from build123d import *

# Parameters (mm, degrees)
SKETCH1_W               = 10.85
SKETCH1_H               = 10.85
BOSS_EXTRUDE1_DEPTH     = 700
MIRROR2_COPY_1_SKETCH_W = 10.85
MIRROR2_COPY_1_SKETCH_H = 10.85
MIRROR2_COPY_1_DEPTH    = 700


with BuildPart() as part:
    # Sketch1 → Boss-Extrude1 (new body)
    with BuildSketch(Plane(origin=(0, 0, 0), x_dir=(1, 0, 0), z_dir=(0, 1, 0))):
        with BuildLine():
            Line((-4.3, 20), (-19.5, 20))
            ThreePointArc((-19.5, 20), (-19.853553391, 19.853553391), (-20, 19.5))
            Line((-20, 19.5), (-20, 4.3))
            Line((-20, 4.3), (-19.05, 4.3))
            Line((-19.05, 4.3), (-19.05, 7.25))
            Line((-19.05, 7.25), (-7.921751442, 7.25))
            Line((-7.921751442, 7.25), (-6.2, 5.528248558))
            Line((-6.2, 5.528248558), (-6.2, 0))
            Line((-6.2, 0), (-5.3, 0))
            ThreePointArc((-5.3, 0), (-5.066731596, 1.555066215), (-4.387460025, 2.973246463))
            Line((-4.387460025, 2.973246463), (-5.091168825, 3.676955262))
            ThreePointArc((-5.091168825, 3.676955262), (-5.091168825, 5.091168825), (-3.676955262, 5.091168825))
            Line((-3.676955262, 5.091168825), (-2.973246463, 4.387460025))
            ThreePointArc((-2.973246463, 4.387460025), (-1.555066215, 5.066731596), (0, 5.3))
            Line((0, 5.3), (0, 6.2))
            Line((0, 6.2), (-5.528248558, 6.2))
            Line((-5.528248558, 6.2), (-7.25, 7.921751442))
            Line((-7.25, 7.921751442), (-7.25, 19.05))
            Line((-7.25, 19.05), (-4.3, 19.05))
            Line((-4.3, 19.05), (-4.3, 20))
        make_face()
        with Locations((-13.625, 13.625)):
            Rectangle(SKETCH1_W, SKETCH1_H, mode=Mode.SUBTRACT)
    boss_extrude1 = extrude(amount=BOSS_EXTRUDE1_DEPTH)

    # Mirror1: Boss-Extrude1 across plane
    add(boss_extrude1.mirror(Plane(origin=(0, 0, 0), x_dir=(0, 0, 1), z_dir=(1, 0, 0))))

    # Mirror2: Boss-Extrude1 across plane
    add(boss_extrude1.mirror(Plane.XY))

    # Mirror2 copy 1 sketch → Mirror2 copy 1 (add)
    with BuildSketch(Plane(origin=(0, 0, 0), x_dir=(-1, 0, 0), z_dir=(0, 1, 0))):
        with BuildLine():
            Line((-4.3, 20), (-19.5, 20))
            ThreePointArc((-19.5, 20), (-19.853553391, 19.853553391), (-20, 19.5))
            Line((-20, 19.5), (-20, 4.3))
            Line((-20, 4.3), (-19.05, 4.3))
            Line((-19.05, 4.3), (-19.05, 7.25))
            Line((-19.05, 7.25), (-7.921751442, 7.25))
            Line((-7.921751442, 7.25), (-6.2, 5.528248558))
            Line((-6.2, 5.528248558), (-6.2, 0))
            Line((-6.2, 0), (-5.3, 0))
            ThreePointArc((-5.3, 0), (-5.066731596, 1.555066215), (-4.387460025, 2.973246463))
            Line((-4.387460025, 2.973246463), (-5.091168825, 3.676955262))
            ThreePointArc((-5.091168825, 3.676955262), (-5.091168825, 5.091168825), (-3.676955262, 5.091168825))
            Line((-3.676955262, 5.091168825), (-2.973246463, 4.387460025))
            ThreePointArc((-2.973246463, 4.387460025), (-1.555066215, 5.066731596), (0, 5.3))
            Line((0, 5.3), (0, 6.2))
            Line((0, 6.2), (-5.528248558, 6.2))
            Line((-5.528248558, 6.2), (-7.25, 7.921751442))
            Line((-7.25, 7.921751442), (-7.25, 19.05))
            Line((-7.25, 19.05), (-4.3, 19.05))
            Line((-4.3, 19.05), (-4.3, 20))
        make_face()
        with Locations((-13.625, 13.625)):
            Rectangle(MIRROR2_COPY_1_SKETCH_W, MIRROR2_COPY_1_SKETCH_H, mode=Mode.SUBTRACT)
    extrude(amount=MIRROR2_COPY_1_DEPTH)


solid = part.part
Design review of the part built by this model. Coordinates are the model's own, in mm. A direction names the side the tool comes from. Give positions to 0.01 mm unless a question says otherwise; leave off trailing zeros. Return JSON: item names as keys, results as strings. Group by question number.
Item 1: Wall thickness on line 1 along X through (y, z) = (176.5, 12.5); line 2 along X through (y, z) = (325, -5.5): over which ranges is each line inside the solid? List them lowest first.
Item 2: Tool access review of faces 4 (the flat face through (0, 700, -6)), 5 (the flat face through (14, 345, -19.05)): name each direction out of +Z, -Z, +X, -X, +Y, -Y from which nothing blocks a thin tool from reaching the whole face with its end or side.
Item 3: Clearance check with flat-ended pins moving along their axes: pin 1 Ø2 at (y, z) = (597.5, 3) entering from +X; pin 2 Ø2 at (x, y) = (0, 414) entering from +Z. State where each tip first meets the part, or that it passes through.
Item 4: Take a section at A-A (y = 319.5). Count the separate pieces of the cut face and the enclosed holes in it, plus the area to 3 significant figures.
Item 5: The part is to be moulded in two halves that separate along X. For faces 1 (the flat face through (-20, 345, 12)), 2 (the flat face through (0, 0, -6)), 3 (the flat face through (7.25, 345, -13)), say which applies: pulls with the +X half, pulls with the -X half, needs draft (parallel to the pull), parting line crosses it, or undercut.
Return value:
{
 "1": {"line 1": "x = -20 to -19.05, -8.2 to -7.25, 7.25 to 8.2, 19.05 to 20", "line 2": "x = -20 to -19.05, -6.2 to 6.2, 19.05 to 20"},
 "2": {"face 4": "+Z, -Z, +X, -X, +Y", "face 5": "+Y, -Y"},
 "3": {"pin 1": "stops at x = 6.2", "pin 2": "stops at z = 6.2"},
 "4": {"separate pieces": "1", "enclosed holes": "5", "area": "261 mm2"},
 "5": {"face 1": "pulls with the -X half", "face 2": "needs draft", "face 3": "undercut"}
}
